Part model, mm, in its own coordinate system. Face numbers are marked on the shaded views. A direction names the side the tool comes from. Round coordinates to 2 decimals unless told otherwise and drop trailing zeros. Loops run counter-clockwise (first coordinate to the right, second up) from the corner with the lowest first, then second, coordinate; pieces in that order, holes last. Notation, with made-up numbers: M 59.25,87.25 L 70.25,87.25 A23 cw 70.25,98.25 Z; hole C 47,77.5 d4. An arc over 180 degrees is marked long. Put each result on its own line as item: value. Start each with the question number.
1) Probe line 1 along X through (y, z) = (27, 7); line 2 along Y through (x, z) = (-6, -3); line 3 along X through (y, z) = (51, 15). List the from-to ranges inside material, lowest first.
2) Which spindle directions (+Z, -Z, +X, -X, +Y, -Y) get a long thin tool onto all of the face, cutting with end or side? Do the marked faces 1, 2, 3 and 4. Say none if no direction does.
3) Slice it at A-A on x = 71. Give the cut face in (y, z), then the cut area to 3 significant figures.
4) Slice it at C-C on y = 7. Give the cut face in (x, z).
5) Slice it at B-B on z = 0. Give the cut face in (x, y).
6) Slice it at D-D on x = -37. Give the cut face in (y, z).
7) Pull direction X, two halves, no side cores. Call the marked faces 5, 6, 7 and 8: +X half, -X half, draft (parallel to the pull), parting line (faces both ways), or undercut.
8) Drop flat-ended pins along their axis: pin 1 Ø9 at (y, z) = (44, -15) entering from +X; pin 2 Ø8.5 at (x, y) = (10.5, 62.5) entering from -Z; pin 3 Ø5.5 at (x, z) = (-64.5, 4) entering from +Y. Give the stop position or say it passes through.
```python
from build123d import *

# Parameters (mm, degrees)
BASE_PLATE_11MM_DEPTH   = 11
CHANNEL_CUT_12X25_DEPTH = 102
BORE_BLOCK_DEPTH        = 50
KEYED_BORE_11_DEPTH     = 68
ANGLED_LUG_DEPTH        = 6
LUG_HOLE_SKETCH_R       = 4.5
LUG_HOLE_9_DEPTH        = 20
END_LUG_SKETCH_W        = 15
END_LUG_SKETCH_H        = 50
END_LUG_DEPTH           = 27
END_LUG_TIP_SKETCH_W    = 10
END_LUG_TIP_SKETCH_H    = 50
END_LUG_TIP_DEPTH       = 16
END_LUG_ROUND_R10_A_R   = 10
END_LUG_ROUND_R10_B_R   = 10
END_LUG_CUT_SKETCH_R    = 3.5
END_LUG_CUT_7_DEPTH     = 16


with BuildPart() as part:
    # Base Plate Sketch → Base Plate 11mm (new body)
    with BuildSketch(Plane(origin=(0, 0, 0), x_dir=(1, 0, 0), z_dir=(0, 1, 0))):
        with BuildLine():
            Line((77.5, -25), (-77.5, -25))
            Line((-77.5, -25), (-77.5, 25))
            Line((-77.5, 25), (77.5, 25))
            ThreePointArc((77.5, 25), (102.5, 0), (77.5, -25))
        make_face()
    extrude(amount=BASE_PLATE_11MM_DEPTH)

    # Channel Cut Sketch → Channel Cut 12x25 (cut)
    with BuildSketch(Plane(origin=(0, 11, 0), x_dir=(1, 0, 0), z_dir=(0, 1, 0))):
        with BuildLine():
            Line((52.5, 12), (77.5, 12))
            ThreePointArc((77.5, 12), (89.5, 0), (77.5, -12))
            Line((77.5, -12), (52.5, -12))
            ThreePointArc((52.5, -12), (40.5, 0), (52.5, 12))
        make_face()
    extrude(amount=-CHANNEL_CUT_12X25_DEPTH, mode=Mode.SUBTRACT)

    # Bore Block Sketch → Bore Block (add)
    with BuildSketch(Plane.XY.offset(25)):
        with BuildLine():
            Line((-24, 11), (13, 11))
            Line((13, 11), (13, 42))
            ThreePointArc((13, 42), (-5.5, 60.5), (-24, 42))
            Line((-24, 42), (-24, 11))
        make_face()
    extrude(amount=-BORE_BLOCK_DEPTH)

    # Keyed Bore Sketch → Keyed Bore Ø11 (cut)
    with BuildSketch(Plane.XY.offset(25)):
        with BuildLine():
            Line((-5.5, 25), (-3, 25))
            Line((-3, 25), (-3, 31.287857357))
            ThreePointArc((-3, 31.287857357), (-5.5, 53), (-8, 31.287857357))
            Line((-8, 31.287857357), (-8, 25))
            Line((-8, 25), (-5.5, 25))
        make_face()
    extrude(amount=-KEYED_BORE_11_DEPTH, mode=Mode.SUBTRACT)

    # Angled Lug Sketch → Angled Lug (add, symmetric)
    with BuildSketch(Plane.XY):
        with BuildLine():
            Line((11.618883443, 49.013831311), (21.045966406, 62.477101054))
            ThreePointArc((21.045966406, 62.477101054), (18.590210327, 76.40438586), (4.66292552, 73.948629781))
            Line((4.66292552, 73.948629781), (-4.764157443, 60.485360038))
            ThreePointArc((-4.764157443, 60.485360038), (5.111164072, 57.154312819), (11.618883443, 49.013831311))
        make_face()
    extrude(amount=ANGLED_LUG_DEPTH, both=True)

    # Lug Hole Sketch → Lug Hole Ø9 (cut)
    with BuildSketch(Plane.XY.offset(6)):
        with Locations((12.854445963, 68.212865417)):
            Circle(LUG_HOLE_SKETCH_R)
    extrude(amount=-LUG_HOLE_9_DEPTH, mode=Mode.SUBTRACT)

    # End Lug Sketch → End Lug (add)
    with BuildSketch(Plane(origin=(0, 11, 0), x_dir=(1, 0, 0), z_dir=(0, 1, 0))):
        with Locations((-70, 0)):
            Rectangle(END_LUG_SKETCH_W, END_LUG_SKETCH_H)
    extrude(amount=END_LUG_DEPTH)

    # End Lug Tip Sketch → End Lug Tip (add)
    with BuildSketch(Plane(origin=(0, 38, 0), x_dir=(1, 0, 0), z_dir=(0, 1, 0))):
        with Locations((-72.5, 0)):
            Rectangle(END_LUG_TIP_SKETCH_W, END_LUG_TIP_SKETCH_H)
    extrude(amount=END_LUG_TIP_DEPTH)

    # End Lug Round R10 A
    end_lug_round_r10_a_edges = [part.edges().sort_by_distance(p)[0] for p in [
        (-72.5, 54, 25),
    ]]
    fillet(end_lug_round_r10_a_edges, radius=END_LUG_ROUND_R10_A_R)

    # End Lug Round R10 B
    end_lug_round_r10_b_edges = [part.edges().sort_by_distance(p)[0] for p in [
        (-72.5, 54, -25),
    ]]
    fillet(end_lug_round_r10_b_edges, radius=END_LUG_ROUND_R10_B_R)

    # End Lug Cut Sketch → End Lug Cut Ø7 (cut)
    with BuildSketch(Plane.ZY.offset(77.5)):
        with Locations((15, 44)):
            Circle(END_LUG_CUT_SKETCH_R)
        with Locations((-15, 44)):
            Circle(END_LUG_CUT_SKETCH_R)
    extrude(amount=-END_LUG_CUT_7_DEPTH, mode=Mode.SUBTRACT)


solid = part.part
```
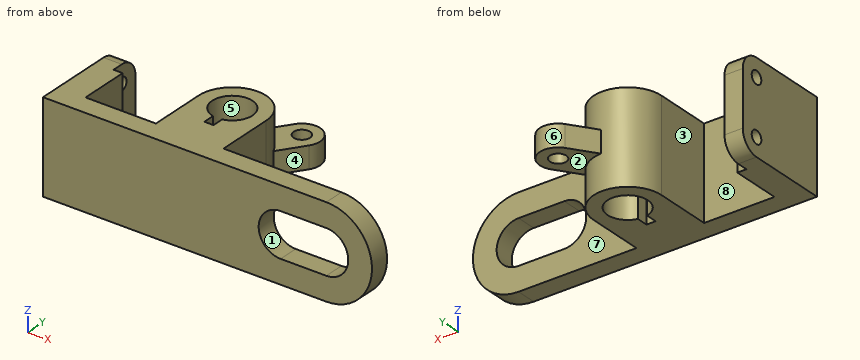
Recorded:
1. line 1: x = -77.5 to -62.5, -24 to -8, -3 to 13
1. line 2: y = 0 to 25, 52.99 to 60.49
1. line 3: x = -77.5 to -67.5, -21.66 to -11.82, 0.82 to 10.66
2. face 1: +Y, -Y
2. face 2: -Z, +X, +Y
2. face 3: +Z, -Z, +Y
2. face 4: +Z, -Z, +X
3. outline: M 0,-25 L 11,-25 L 11,-12 L 0,-12 Z; M 0,12 L 11,12 L 11,25 L 0,25 Z
3. area: 286 mm2
4. outline: M -77.5,-25 L 77.5,-25 A25 ccw 77.5,25 L -77.5,25 Z; hole M 52.5,-12 L 77.5,-12 A12 ccw 77.5,12 L 52.5,12 A12 ccw Z
5. outline: M -77.5,0 L 40.5,0 L 40.5,11 L 13,11 L 13,42 A18.5 ccw 11.62,49.01 L 21.05,62.48 A10 ccw 4.66,73.95 L -4.76,60.49 A18.5 ccw -24,42 L -24,11 L -62.5,11 L -62.5,38 L -67.5,38 L -67.5,54 L -77.5,54 Z; M 89.5,0 L 102.5,0 L 102.5,11 L 89.5,11 Z; hole M -8,25 L -3,25 L -3,31.29 A11 ccw long -8,31.29 Z; hole C 12.85,68.21 d9
6. outline: M 0,-25 L 11,-25 L 11,25 L 0,25 Z
7. face 5: undercut
7. face 6: parting line
7. face 7: draft
7. face 8: undercut
8. pin 1: stops at x = 13
8. pin 2: stops at z = -6
8. pin 3: stops at y = 38
